```python
from build123d import *

# Parameters (mm, degrees)
SKETCH_1_W                     = 390
SKETCH_1_H                     = 225
EXTRUDE_1_DEPTH                = 40
FILLET_1_R                     = 20
SHELL_1_T                      = -3
FILLET_2_R                     = 2
SKETCH_2_R                     = 7.5
EXTRUDE_2_DEPTH                = 8
FILLET_3_R                     = 2
PATTERN_LINEAR_1_COUNT         = 2
PATTERN_LINEAR_1_PITCH         = 260
PATTERN_LINEAR_1_COUNT_DIR2    = 2
PATTERN_LINEAR_1_PITCH_DIR2    = 130
FILLET_3_OF_PATTERN_LINEAR_1_R = 2


with BuildPart() as part:
    # 草图1 → 凸台-拉伸1 (new body)
    with BuildSketch(Plane.XY):
        Rectangle(SKETCH_1_W, SKETCH_1_H)
    extrude(amount=EXTRUDE_1_DEPTH)

    # 圆角1
    fillet_1_edges = [part.edges().sort_by_distance(p)[0] for p in [
        (195, -112.5, 20),
        (-195, -112.5, 20),
        (-195, 112.5, 20),
        (195, 112.5, 20),
    ]]
    fillet(fillet_1_edges, radius=FILLET_1_R)

    # 抽壳1
    shell_1_openings = [part.faces().sort_by_distance(p)[0] for p in [
        (0, 0, 40),
    ]]
    offset(amount=SHELL_1_T, openings=shell_1_openings, kind=Kind.INTERSECTION)

    # 圆角2
    fillet_2_edges = [part.edges().sort_by_distance(p)[0] for p in [
        (195, 0, 0),
        (0, -112.5, 0),
        (-195, 0, 0),
        (0, 112.5, 0),
        (-189.142135624, -106.642135624, 0),
        (189.142135624, 106.642135624, 0),
        (-189.142135624, 106.642135624, 0),
        (189.142135624, -106.642135624, 0),
    ]]
    fillet(fillet_2_edges, radius=FILLET_2_R)

    # 草图2 → 凸台-拉伸2 (add)
    with BuildSketch(Plane(origin=(0, 0, 0), x_dir=(-1, 0, 0), z_dir=(0, 0, -1))):
        with Locations((-130, 65)):
            Circle(SKETCH_2_R)
    extrude_2 = extrude(amount=EXTRUDE_2_DEPTH)

    # 圆角3
    fillet_3_edges = [part.edges().sort_by_distance(p)[0] for p in [
        (137.5, 65, -8),
    ]]
    fillet(fillet_3_edges, radius=FILLET_3_R)

    # 阵列(线性)1: Extrude 2 2 × 2
    with Locations(*[(-i * PATTERN_LINEAR_1_PITCH, -j * PATTERN_LINEAR_1_PITCH_DIR2, 0) for i in range(PATTERN_LINEAR_1_COUNT) for j in range(PATTERN_LINEAR_1_COUNT_DIR2) if (i, j) != (0, 0)]):
        add(extrude_2)

    # 圆角3 of 阵列(线性)1
    fillet_3_of_pattern_linear_1_edges = [part.edges().sort_by_distance(p)[0] for p in [
        (137.5, -65, -8),
        (-122.5, 65, -8),
        (-122.5, -65, -8),
    ]]
    fillet(fillet_3_of_pattern_linear_1_edges, radius=FILLET_3_OF_PATTERN_LINEAR_1_R)


solid = part.part
```
Design review of the part built by this model. Coordinates are the model's own, in mm. A direction names the side the tool comes from. Coordinates: 2 decimals unless noted, no trailing zeros. Order: outer loops, then holes, each group sorted by start corner. A loop starts at its lowest first (then second) coordinate and runs counter-clockwise, first axis right, second up.
1) Take a section at B-B, the plane z = 22.5. Give the boundary of the cut face in (x, y), and give its area (3 significant figures).
2) Mouldability with a two-part tool opening along Y and no side actions: class faces 4 (the flat face through (130, 65, -8)), 5 (the cylindrical face through (-189.297, -106.486, 21.266)), 6 (the flat face through (-2, 112.5, 21)), 7 (the cylindrical face through (-187.15, -104.39, 21.76)) as +Y half, -Y half, draft (parallel to the pull), parting line (faces both ways), or undercut.
3) Take a section at D-D, the plane x = -130. Give the boundary of the cut face in (y, z).
4) Take a section at A-A, the plane y = -87. Give the boundary of the cut face in (x, z), and give its area (3 significant figures).
5) Take a section at C-C, the plane x = 170.5. Give the boundary of the cut face in (y, z).
6) Wall thickness on line 1 along X through (y, z) = (26.5, 16); line 2 along Y through (x, z) = (-22, 8); line 3 along Y through (x, z) = (-125, -1): over which ranges is each line inside the solid? List them lowest first.
7) For faces 1 (the cylindrical face through (-137.154, 67.253, -2.958)), 2 (the cylindrical face through (-187.15, 104.39, 21.76)), 3 (the flat face through (-2, -112.5, 21)), list the 3-axis set-ups (+Z, -Z, +X, -X, +Y, -Y) from which the entire face can be reached by the end or side of a thin tool; tool diameter is ignored.
8) Clearance check with flat-ended pins moving along their axes: pin 1 (6 mm diameter, centred on x = 109, y = -74.5, fed in from +Z); pin 2 (8 mm diameter, centred on x = 141, y = 57, fed in from -Z). State where each tip first meets the part, or that it passes through.
Returned:
1. outline: (-195, -92.5) arc R20 ccw to (-175, -112.5) - (175, -112.5) arc R20 ccw to (195, -92.5) - (195, 92.5) arc R20 ccw to (175, 112.5) - (-175, 112.5) arc R20 ccw to (-195, 92.5) - close; hole (-192, -92.5) arc R17 ccw to (-175, -109.5) - (175, -109.5) arc R17 ccw to (192, -92.5) - (192, 92.5) arc R17 ccw to (175, 109.5) - (-175, 109.5) arc R17 ccw to (-192, 92.5) - close
1. area: 3,560 mm2
2. face 4: draft
2. face 5: -Y half
2. face 6: +Y half
2. face 7: undercut
3. outline: (-112.5, 2) arc R2 ccw to (-110.5, 0) - (-72.5, 0) - (-72.5, -6) arc R2 ccw to (-70.5, -8) - (-59.5, -8) arc R2 ccw to (-57.5, -6) - (-57.5, 0) - (57.5, 0) - (57.5, -6) arc R2 ccw to (59.5, -8) - (70.5, -8) arc R2 ccw to (72.5, -6) - (72.5, 0) - (110.5, 0) arc R2 ccw to (112.5, 2) - (112.5, 40) - (109.5, 40) - (109.5, 3) - (-109.5, 3) - (-109.5, 40) - (-112.5, 40) - close
4. outline: (-195, 2) arc R2 ccw to (-193, 0) - (193, 0) arc R2 ccw to (195, 2) - (195, 40) - (192, 40) - (192, 3) - (-192, 3) - (-192, 40) - (-195, 40) - close
4. area: 1,390 mm2
5. outline: (-112.5, 2) arc R2 ccw to (-110.5, 0) - (110.5, 0) arc R2 ccw to (112.5, 2) - (112.5, 40) - (109.5, 40) - (109.5, 3) - (-109.5, 3) - (-109.5, 40) - (-112.5, 40) - close
6. line 1: x = -195 to -192, 192 to 195
6. line 2: y = -112.5 to -109.5, 109.5 to 112.5
6. line 3: y = -70.59 to -59.41, 59.41 to 70.59
7. face 1: -Z
7. face 2: +Z
7. face 3: +Z, -Z, +X, -X, -Y
8. pin 1: stops at z = 3
8. pin 2: stops at z = 0
